Design review of the part shown in the three views and the two pictorial views. Dimensions are in mm from the part's minimum x, y and z. Give positions to 0.01 mm unless a question says otherwise; leave off trailing zeros. Order: outer loops, then holes, each group sorted by start corner. A loop starts at its lowest first (then second) coordinate and runs counter-clockwise, first axis right, second up. Notation, with made-up numbers: (35, 19.5) -> (76, 19.5) arc R19 ccw to (76, 37.5) -> close; hole circle Ø4 at (-4, 29.25). An arc over 180 degrees is marked (long way). Answer in a Markdown table with one row per item. Add a question column.
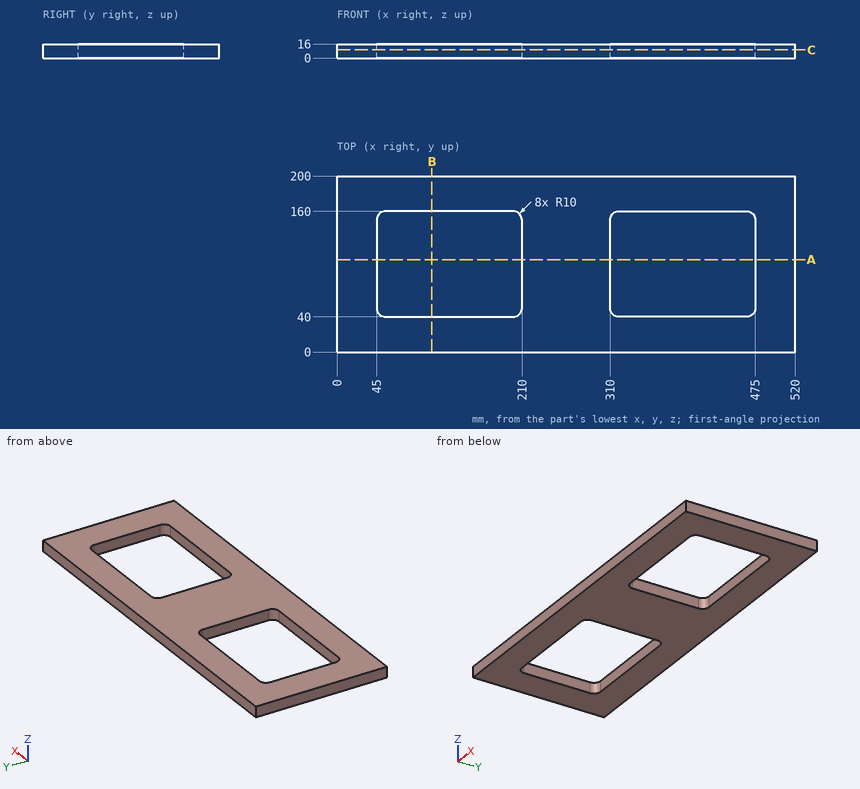
1) Add section B-B, the plane x = 107.5. Write out the cut boundary in (y, z), and give its area (3 significant figures).
2) Add section C-C, the plane z = 9.25. Write out the cut boundary in (x, y).
3) Add section A-A, the plane y = 105. Write out the cut boundary in (x, z).
4) For L1, parallel to X at y = 69.5, z = 15.25; L2, parallel to X at y = 154, z = 2; L3, parallel to Y at x = 411, z = 12.75, list the stretches that pass through material, from the lowest coordinate up.
5) Clearance check with a flat-ended pin moving along its axis: P1, Ø5, axis at y = 94, z = 6.5, coming from the -X side. State where the tip first meets the part, or that it passes through.
Verdict:
| question | item | result |
|---|---|---|
| 1 | outline | (0, 0) -> (40, 0) -> (40, 16) -> (0, 16) -> close; (160, 0) -> (200, 0) -> (200, 16) -> (160, 16) -> close |
| 1 | area | 1,280 mm2 |
| 2 | outline | (0, 0) -> (520, 0) -> (520, 200) -> (0, 200) -> close; hole (45, 50) arc R10 ccw to (55, 40) -> (200, 40) arc R10 ccw to (210, 50) -> (210, 150) arc R10 ccw to (200, 160) -> (55, 160) arc R10 ccw to (45, 150) -> close; hole (310, 50) arc R10 ccw to (320, 40) -> (465, 40) arc R10 ccw to (475, 50) -> (475, 150) arc R10 ccw to (465, 160) -> (320, 160) arc R10 ccw to (310, 150) -> close |
| 3 | outline | (0, 0) -> (45, 0) -> (45, 16) -> (0, 16) -> close; (210, 0) -> (310, 0) -> (310, 16) -> (210, 16) -> close; (475, 0) -> (520, 0) -> (520, 16) -> (475, 16) -> close |
| 4 | L1 | x = 0 to 45, 210 to 310, 475 to 520 |
| 4 | L2 | x = 0 to 45.83, 209.17 to 310.83, 474.17 to 520 |
| 4 | L3 | y = 0 to 40, 160 to 200 |
| 5 | P1 | stops at x = 0 |
